```python
from build123d import *

# Parameters (mm, degrees)
SKETCH_1_W             = 15
SKETCH_1_H             = 18
EXTRUDE_1_DEPTH        = 30
SKETCH_2_R             = 3
CUT_EXTRUDE_1_DEPTH    = 39.065732621
CUT_EXTRUDE_3_DEPTH    = 3
PATTERN_LINEAR_1_COUNT = 2
PATTERN_LINEAR_1_PITCH = 20
SKETCH_5_W             = 6
SKETCH_5_H             = 12.5
CUT_EXTRUDE_4_DEPTH    = 3


with BuildPart() as part:
    # 草图1 → 拉伸1 (new body)
    with BuildSketch(Plane.XY):
        with Locations((7.5, 9)):
            Rectangle(SKETCH_1_W, SKETCH_1_H)
    extrude(amount=EXTRUDE_1_DEPTH)

    # 草图2 → 切除-拉伸1 (cut, through all)
    with BuildSketch(Plane(origin=(0, 18, 0), x_dir=(-1, 0, 0), z_dir=(0, 1, 0))):
        with Locations(Location((-6, 5, 0), (0, 0, 90))):
            Circle(SKETCH_2_R)
    cut_extrude_1 = extrude(amount=-CUT_EXTRUDE_1_DEPTH, mode=Mode.SUBTRACT)

    # 草图4 → 切除-拉伸3 (cut)
    with BuildSketch(Plane(origin=(0, 18, 0), x_dir=(-1, 0, 0), z_dir=(0, 1, 0))):
        with BuildLine():
            Line((-15, 2), (-6, 2))
            ThreePointArc((-6, 2), (-3, 5), (-6, 8))
            Line((-6, 8), (-15, 8))
            Line((-15, 8), (-15, 2))
        make_face()
    cut_extrude_3 = extrude(amount=-CUT_EXTRUDE_3_DEPTH, mode=Mode.SUBTRACT)

    # 阵列(线性)1: 切除-拉伸1, 切除-拉伸3 ×2
    with Locations(*[(0, 0, i * PATTERN_LINEAR_1_PITCH) for i in range(1, PATTERN_LINEAR_1_COUNT)]):
        add(cut_extrude_1, mode=Mode.SUBTRACT)
        add(cut_extrude_3, mode=Mode.SUBTRACT)

    # 草图5 → 切除-拉伸4 (cut)
    with BuildSketch(Plane(origin=(15, 3, 0), x_dir=(0, 1, 0), z_dir=(-1, 0, 0))):
        with Locations((12, -15)):
            Rectangle(SKETCH_5_W, SKETCH_5_H)
    extrude(amount=CUT_EXTRUDE_4_DEPTH, mode=Mode.SUBTRACT)


solid = part.part
```
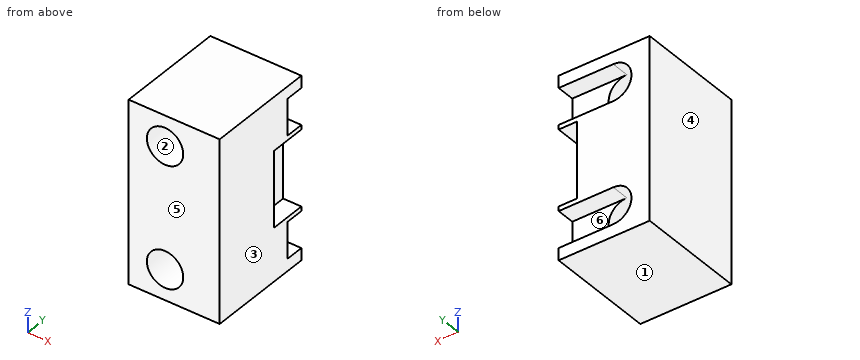
CAD build for the part. Positions are in the model's coordinates, mm. Face numbers are marked on the shaded views. A direction names the side the tool comes from. Round coordinates to 2 decimals unless told otherwise and drop trailing zeros. Write each loop counter-clockwise with the first axis right and the second up, starting at its lowest first coordinate (ties: lowest second). Pieces come first, ordered by that corner, then holes. Notation, with made-up numbers: (41, -1) - (76, -1) arc R17 cw to (76, 31) - close; hole circle Ø10 at (85, 55.5). An arc over 180 degrees is marked (long way). Return JSON: item names as keys, results as strings. Group by question number.
Item 1: Probe probe 1 along Z at (x, y) = (6, 9.5); probe 2 along X at (y, z) = (10.5, 25); probe 3 along Z at (x, y) = (8, 11.5). List the from-to ranges inside material, lowest first.
Item 2: Mould opens along X. For the marked faces 1, 2, 3 and 4 say: +X half, -X half, draft (parallel to the pull), parting line (faces both ways), or undercut.
Item 3: Flat gauge pins, fed straight in: pin 1 Ø3.5 at (x, z) = (6, 5) entering from -Y; pin 2 Ø2.5 at (x, z) = (13, 16.5) entering from +Y; pin 3 Ø1.8 at (x, z) = (11.5, 4) entering from +Y; pin 4 Ø1.8 at (y, z) = (16, 17) entering from +X. Where does each tip first touch, or does it go through?
Item 4: Band-saw the part on B-B on z = 5. List the corners of the cut face in (x, y).
Item 5: 3-axis set-ups, long thin cutter, end or side, ignore diameter. For the marked faces 5 and 6: which of +Z, -Z, +X, -X, +Y, -Y reach the whole face in a straight line?
Item 6: Band-saw the part on D-D on y = 15.75. List the corners of the cut face in (x, z), plus the area to 3 significant figures.
Item 7: Band-saw the part on C-C on y = 6. List the corners of the cut face in (x, z).
Item 8: Band-saw the part on A-A on x = 5. List the corners of the cut face in (y, z).
Resolved:
{
 "1": {"probe 1": "z = 0 to 2, 8 to 22, 28 to 30", "probe 2": "x = 0 to 3, 9 to 15", "probe 3": "z = 0 to 2.76, 7.24 to 22.76, 27.24 to 30"},
 "2": {"face 1": "draft", "face 2": "undercut", "face 3": "+X half", "face 4": "-X half"},
 "3": {"pin 1": "passes through", "pin 2": "stops at y = 18", "pin 3": "stops at y = 15", "pin 4": "stops at x = 12"},
 "4": {"outline": "(0, 0) - (3, 0) - (3, 18) - (0, 18) - close; (9, 0) - (15, 0) - (15, 15) - (9, 15) - close"},
 "5": {"face 5": "+Z, -Z, +X, -X, -Y", "face 6": "+X, +Y"},
 "6": {"outline": "(0, 0) - (15, 0) - (15, 2) - (6, 2) arc R3 cw to (6, 8) - (15, 8) - (15, 8.75) - (12, 8.75) - (12, 21.25) - (15, 21.25) - (15, 22) - (6, 22) arc R3 cw to (6, 28) - (15, 28) - (15, 30) - (0, 30) - close", "area": "276 mm²"},
 "7": {"outline": "(0, 0) - (15, 0) - (15, 30) - (0, 30) - close; hole circle Ø6 at (6, 5); hole circle Ø6 at (6, 25)"},
 "8": {"outline": "(0, 0) - (18, 0) - (18, 2.17) - (0, 2.17) - close; (0, 7.83) - (18, 7.83) - (18, 22.17) - (0, 22.17) - close; (0, 27.83) - (18, 27.83) - (18, 30) - (0, 30) - close"}
}
